Could you check a few things on this model? Use its own coordinates, in mm. A direction names the side the tool comes from. Coordinates: 2 decimals unless noted, no trailing zeros. Loops run counter-clockwise (first coordinate to the right, second up) from the corner with the lowest first, then second, coordinate; pieces in that order, holes last.
1) Thinking about a two-plate mould opening in X: for faces 1 (the face through (36.685, -2.363, -0.616)), 2 (the face through (38.227, 9.85, 0.154)), 3 (the face through (0.546, 11.746, -14.748)), 4 (the face through (-38.98, 0, 0)), which applies, released by +X, released by -X, zero draft, split by the parting line, or undercut?
2) If I drill on line 1 along Z through (x, y) = (-34.73, 10.05); line 2 along Z through (x, y) = (34.73, -8.5); line 3 along Y through (x, z) = (31.5, -0.5) (3 decimals), over which ranges is the centre line in solid material (lowest first)?
3) Imagine slicing it at B-B on x = 34.73. Please give me the cut outline in (y, z) (3 decimals).
4) Imagine slicing it at C-C on y = 9. Please give me the cut outline in (x, z), plus the area to 3 significant figures.
5) Will these pins go through, and if not, where does the flat tip stop? P1, Ø4.5, axis at x = 34.73, z = 0, coming from the -Y side (3 decimals); P2, Ø5.5, axis at x = 34.73, z = 0, coming from the +Y side (3 decimals).
6) Imagine slicing it at A-A on z = 0. Please give me the cut outline in (x, y) (3 decimals).
7) For faces 5 (the face through (33, 7.315, -2)), 6 (the face through (-1, -12.315, 0)), which set-ups out of +Z, -Z, +X, -X, +Y, -Y let a thin tool reach every point of the face, with its end or its side?
```python
from build123d import *

# Parameters (mm, degrees)
SKETCH_1_W          = 77.96
SKETCH_1_H          = 24.63
EXTRUDE_1_DEPTH     = 18.7
CUT_EXTRUDE_1_DEPTH = 82.111718173
SKETCH_3_R          = 2.05
CUT_EXTRUDE_2_DEPTH = 50.757082913
SKETCH_4_R          = 3.5
CUT_EXTRUDE_3_DEPTH = 5


with BuildPart() as part:
    # 草图1 → 凸台-拉伸1 (new, symmetric)
    with BuildSketch(Plane.XY):
        Rectangle(SKETCH_1_W, SKETCH_1_H)
    extrude(amount=EXTRUDE_1_DEPTH, both=True)

    # 草图2 → 切除-拉伸1 (cut, through all)
    with BuildSketch(Plane(origin=(38.98, 0, 0), x_dir=(0, 0, -1), z_dir=(1, 0, 0))):
        with BuildLine():
            Line((-18.7, 10.315), (-18.7, 12.315))
            Line((-18.7, 12.315), (-10.7, 12.315))
            ThreePointArc((-10.7, 12.315), (-14.804196751, 11.731787003), (-18.7, 10.315))
        make_face()
        with BuildLine():
            Line((18.7, 12.315), (10.7, 12.315))
            ThreePointArc((10.7, 12.315), (14.804196751, 11.731787003), (18.7, 10.315))
            Line((18.7, 10.315), (18.7, 12.315))
        make_face()
    extrude(amount=-CUT_EXTRUDE_1_DEPTH, mode=Mode.SUBTRACT)

    # 草图3 → 切除-拉伸2 (cut, through all)
    with BuildSketch(Plane(origin=(0, 12.315, 0), x_dir=(1, 0, 0), z_dir=(0, 1, 0))):
        with Locations(Location((-34.73, 0, 0), (0, 0, 180))):
            Circle(SKETCH_3_R)
        with Locations((34.73, 0)):
            Circle(SKETCH_3_R)
    extrude(amount=-CUT_EXTRUDE_2_DEPTH, mode=Mode.SUBTRACT)

    # 草图4 → 切除-拉伸3 (cut)
    with BuildSketch(Plane(origin=(0, 12.315, 0), x_dir=(1, 0, 0), z_dir=(0, 1, 0))):
        with Locations(Location((-34.73, 0, 0), (0, 0, 180))):
            Circle(SKETCH_4_R)
        with Locations(Location((34.73, 0, 0), (0, 0, 180))):
            Circle(SKETCH_4_R)
    extrude(amount=-CUT_EXTRUDE_3_DEPTH, mode=Mode.SUBTRACT)


solid = part.part
```
Filled in:
1. face 1: undercut
1. face 2: undercut
1. face 3: zero draft
1. face 4: released by -X
2. line 1: z = -18.7 to -3.5, 3.5 to 18.7
2. line 2: z = -18.7 to -2.05, 2.05 to 18.7
2. line 3: y = -12.315 to 7.315
3. outline: (-12.315, -18.7) - (10.315, -18.7) arc R20 ccw to (12.315, -10.7) - (12.315, -3.5) - (7.315, -3.5) - (7.315, -2.05) - (-12.315, -2.05) - close; (-12.315, 2.05) - (7.315, 2.05) - (7.315, 3.5) - (12.315, 3.5) - (12.315, 10.7) arc R20 ccw to (10.315, 18.7) - (-12.315, 18.7) - close
4. outline: (-38.98, -18.7) - (38.98, -18.7) - (38.98, 18.7) - (-38.98, 18.7) - close; hole circle Ø7 at (-34.73, 0); hole circle Ø7 at (34.73, 0)
4. area: 2,840 mm2
5. P1: stops at y = -12.315
5. P2: stops at y = 7.315
6. outline: (-38.98, -12.315) - (-36.78, -12.315) - (-36.78, 7.315) - (-38.23, 7.315) - (-38.23, 12.315) - (-38.98, 12.315) - close; (-32.68, -12.315) - (32.68, -12.315) - (32.68, 7.315) - (31.23, 7.315) - (31.23, 12.315) - (-31.23, 12.315) - (-31.23, 7.315) - (-32.68, 7.315) - close; (36.78, -12.315) - (38.98, -12.315) - (38.98, 12.315) - (38.23, 12.315) - (38.23, 7.315) - (36.78, 7.315) - close
7. face 5: +Y
7. face 6: +Z, -Z, +X, -X, -Y
